```python
from build123d import *

# Parameters (mm, degrees)
BASE_BLOCK_SKETCH_W              = 200
BASE_BLOCK_SKETCH_H              = 160
BASE_BLOCK_DEPTH                 = 50
BEARING_HOUSING_DEPTH            = 50
BASE_RELIEF_CUT_SKETCH_W         = 100
BASE_RELIEF_CUT_SKETCH_H         = 100
BASE_RELIEF_CUT_DEPTH            = 50
BEARING_BORE_SKETCH_R            = 65
BEARING_BORE_DEPTH_35_DEPTH      = 35
FORK_SLOT_DEPTH                  = 200
UPPER_ARM_DEPTH                  = 30
UPPER_START                      = -30
UPPER_ARM_LUG_DEPTH              = 30
UPPER_LUG_COUNTERBORE_SKETCH_R   = 18
UPPER_LUG_COUNTERBORE_36X5_DEPTH = 5
UPPER_LUG_HOLE_SKETCH_R          = 7
UPPER_LUG_HOLE_14_DEPTH          = 50
UPPER_START_2                    = -5
UPPER_ARM_COUNTERBORE_SKETCH_R   = 18
UPPER_ARM_COUNTERBORE_36X5_DEPTH = 5
UPPER_START_3                    = -50
UPPER_ARM_HOLE_SKETCH_R          = 7
UPPER_ARM_HOLE_14_DEPTH          = 50
LOWER_ARM_DEPTH                  = 30
LOWER_START                      = -30
LOWER_ARM_LUG_DEPTH              = 30
LOWER_ARM_COUNTERBORE_SKETCH_R   = 18
LOWER_ARM_COUNTERBORE_36X5_DEPTH = 5
LOWER_ARM_HOLE_SKETCH_R          = 10
LOWER_ARM_HOLE_20_DEPTH          = 40
CROSS_HOLE_SKETCH_R              = 10
CROSS_HOLE_20_DEPTH              = 160
LOWER_START_2                    = -5
LOWER_LUG_COUNTERBORE_SKETCH_R   = 18
LOWER_LUG_COUNTERBORE_36X5_DEPTH = 5
LOWER_LUG_HOLE_SKETCH_R          = 10
LOWER_LUG_HOLE_20_DEPTH          = 30
SHAFT_BORE_SKETCH_R              = 25
SHAFT_BORE_50_DEPTH              = 30


with BuildPart() as part:
    # Base Block Sketch → Base Block (new body)
    with BuildSketch(Plane.XY):
        with Locations((100, 80)):
            Rectangle(BASE_BLOCK_SKETCH_W, BASE_BLOCK_SKETCH_H)
    extrude(amount=BASE_BLOCK_DEPTH)

    # Bearing Housing Sketch → Bearing Housing (add)
    with BuildSketch(Plane.XY.offset(50)):
        with BuildLine():
            Line((0, 160), (0, 0))
            ThreePointArc((0, 0), (-80, 80), (0, 160))
        make_face()
    extrude(amount=-BEARING_HOUSING_DEPTH)

    # Base Relief Cut Sketch → Base Relief Cut (cut)
    with BuildSketch(Plane.XY.offset(50)):
        with Locations((150, 80)):
            Rectangle(BASE_RELIEF_CUT_SKETCH_W, BASE_RELIEF_CUT_SKETCH_H)
    extrude(amount=-BASE_RELIEF_CUT_DEPTH, mode=Mode.SUBTRACT)

    # Bearing Bore Sketch → Bearing Bore Depth 35 (cut)
    with BuildSketch(Plane.XY.offset(50)):
        with Locations((0, 80)):
            Circle(BEARING_BORE_SKETCH_R)
    extrude(amount=-BEARING_BORE_DEPTH_35_DEPTH, mode=Mode.SUBTRACT)

    # Fork Slot Sketch → Fork Slot (cut)
    with BuildSketch(Plane(origin=(100, 0, 0), x_dir=(0, 0, -1), z_dir=(1, 0, 0))):
        Polygon((-50, 80), (-50, 90), (-35, 90), (-35, 70), (-50, 70), align=None)
    extrude(amount=-FORK_SLOT_DEPTH, mode=Mode.SUBTRACT)

    # Upper Arm Sketch → Upper Arm (add)
    with BuildSketch(Plane.XZ):
        with BuildLine():
            Line((125, 0), (100, 0))
            Line((100, 0), (75, 0))
            Line((75, 0), (75, -36.5))
            ThreePointArc((75, -36.5), (100, -61.5), (125, -36.5))
            Line((125, -36.5), (125, 0))
        make_face()
    extrude(amount=-UPPER_ARM_DEPTH)

    # Upper Arm Lug Sketch → Upper Arm Lug (add)
    with BuildSketch(Plane(origin=(0, 160, 0), x_dir=(1, 0, 0), z_dir=(0, 1, 0)).offset(UPPER_START)):
        with BuildLine():
            Line((75, 36.5), (75, 0))
            Line((75, 0), (125, 0))
            Line((125, 0), (125, 36.5))
            ThreePointArc((125, 36.5), (100, 61.5), (75, 36.5))
        make_face()
    extrude(amount=UPPER_ARM_LUG_DEPTH)

    # Upper Lug Counterbore Sketch → Upper Lug Counterbore Ø36x5 (cut)
    with BuildSketch(Plane(origin=(0, 160, 0), x_dir=(1, 0, 0), z_dir=(0, 1, 0))):
        with Locations(Location((100, 36.5, 0), (0, 0, 270))):
            Circle(UPPER_LUG_COUNTERBORE_SKETCH_R)
    extrude(amount=-UPPER_LUG_COUNTERBORE_36X5_DEPTH, mode=Mode.SUBTRACT)

    # Upper Lug Hole Sketch → Upper Lug Hole Ø14 (cut)
    with BuildSketch(Plane(origin=(0, 155, 0), x_dir=(1, 0, 0), z_dir=(0, 1, 0))):
        with Locations(Location((100, 36.5, 0), (0, 0, 270))):
            Circle(UPPER_LUG_HOLE_SKETCH_R)
    extrude(amount=-UPPER_LUG_HOLE_14_DEPTH, mode=Mode.SUBTRACT)

    # Upper Arm Counterbore Sketch → Upper Arm Counterbore Ø36x5 (cut)
    with BuildSketch(Plane.XZ.offset(UPPER_START_2)):
        with Locations(Location((100, -36.5, 0), (0, 0, 90))):
            Circle(UPPER_ARM_COUNTERBORE_SKETCH_R)
    extrude(amount=UPPER_ARM_COUNTERBORE_36X5_DEPTH, mode=Mode.SUBTRACT)

    # Upper Arm Hole Sketch → Upper Arm Hole Ø14 (cut)
    with BuildSketch(Plane.XZ.offset(-5).offset(UPPER_START_3)):
        with Locations(Location((100, -36.5, 0), (0, 0, 90))):
            Circle(UPPER_ARM_HOLE_SKETCH_R)
    extrude(amount=UPPER_ARM_HOLE_14_DEPTH, mode=Mode.SUBTRACT)

    # Lower Arm Sketch → Lower Arm (add)
    with BuildSketch(Plane.XZ):
        with BuildLine():
            Line((225, 25), (200, 25))
            Line((200, 25), (200, 50))
            ThreePointArc((200, 50), (182.32233047, 7.32233047), (225, 25))
        make_face()
    extrude(amount=-LOWER_ARM_DEPTH)

    # Lower Arm Lug Sketch → Lower Arm Lug (add)
    with BuildSketch(Plane(origin=(0, 160, 0), x_dir=(1, 0, 0), z_dir=(0, 1, 0)).offset(LOWER_START)):
        with BuildLine():
            Line((200, -25), (225, -25))
            ThreePointArc((225, -25), (217.67766953, -7.32233047), (200, 0))
            Line((200, 0), (200, -25))
        make_face()
    extrude(amount=LOWER_ARM_LUG_DEPTH)

    # Lower Arm Counterbore Sketch → Lower Arm Counterbore Ø36x5 (cut)
    with BuildSketch(Plane.XZ):
        with Locations((200, 25)):
            Circle(LOWER_ARM_COUNTERBORE_SKETCH_R)
    extrude(amount=-LOWER_ARM_COUNTERBORE_36X5_DEPTH, mode=Mode.SUBTRACT)

    # Lower Arm Hole Sketch → Lower Arm Hole Ø20 (cut)
    with BuildSketch(Plane.XZ.offset(-5)):
        with Locations((200, 25)):
            Circle(LOWER_ARM_HOLE_SKETCH_R)
    extrude(amount=-LOWER_ARM_HOLE_20_DEPTH, mode=Mode.SUBTRACT)

    # Cross Hole Sketch → Cross Hole Ø20 (cut)
    with BuildSketch(Plane.XZ.offset(-5)):
        with Locations(Location((100, -36.5, 0), (0, 0, 270))):
            Circle(CROSS_HOLE_SKETCH_R)
    extrude(amount=-CROSS_HOLE_20_DEPTH, mode=Mode.SUBTRACT)

    # Lower Lug Counterbore Sketch → Lower Lug Counterbore Ø36x5 (cut)
    with BuildSketch(Plane(origin=(0, 160, 0), x_dir=(1, 0, 0), z_dir=(0, 1, 0)).offset(LOWER_START_2)):
        with Locations((200, -25)):
            Circle(LOWER_LUG_COUNTERBORE_SKETCH_R)
    extrude(amount=LOWER_LUG_COUNTERBORE_36X5_DEPTH, mode=Mode.SUBTRACT)

    # Lower Lug Hole Sketch → Lower Lug Hole Ø20 (cut)
    with BuildSketch(Plane(origin=(0, 160, 0), x_dir=(1, 0, 0), z_dir=(0, 1, 0)).offset(LOWER_START)):
        with Locations((200, -25)):
            Circle(LOWER_LUG_HOLE_SKETCH_R)
    extrude(amount=LOWER_LUG_HOLE_20_DEPTH, mode=Mode.SUBTRACT)

    # Shaft Bore Sketch → Shaft Bore Ø50 (cut)
    with BuildSketch(Plane.XY.offset(15)):
        with Locations((0, 80)):
            Circle(SHAFT_BORE_SKETCH_R)
    extrude(amount=-SHAFT_BORE_50_DEPTH, mode=Mode.SUBTRACT)


solid = part.part
```
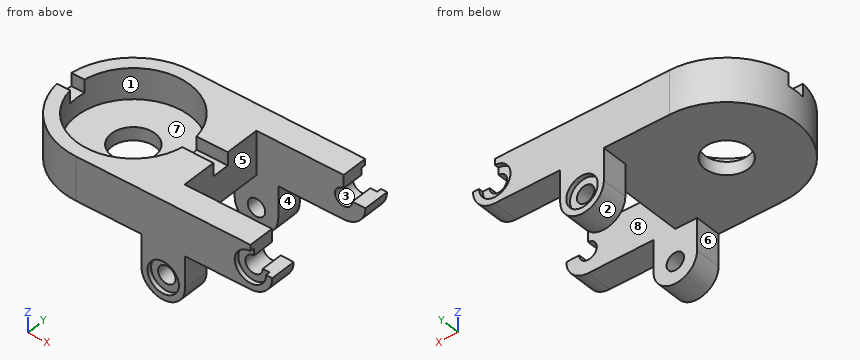
Part model, mm, in its own coordinate system. Face numbers are marked on the shaded views. A direction names the side the tool comes from. Round coordinates to 2 decimals unless told otherwise and drop trailing zeros. Order: outer loops, then holes, each group sorted by start corner. A loop starts at its lowest first (then second) coordinate and runs counter-clockwise, first axis right, second up. Notation, with made-up numbers: M 12,7 L 28,7 A23 ccw 28,22 Z; hole C -12,20 d2. An arc over 180 degrees is marked long. Put each result on its own line as item: value. Start each with the question number.
1. Slice it at B-B on x = 171. List the corners of the cut face in (y, z), then the cut area to 3 significant figures.
2. Slice it at C-C on z = 29.5. List the corners of the cut face in (x, y), then the cut area to 3 significant figures.
3. Slice it at D-D on y = 110. List the corners of the cut face in (x, z), then the cut area to 3 significant figures.
4. Drop flat-ended pins along their axis: pin 1 (4 mm diameter, centred on x = -37.5, y = 98.5, fed in from -Z); pin 2 (7.5 mm diameter, centred on x = 215.5, y = 13, fed in from +Z); pin 3 (2 mm diameter, centred on y = 18.5, z = -18, fed in from +X). Give the stop position or say it passes through.
5. Slice it at A-A on y = 80. List the corners of the cut face in (x, z).
6. Tool access for the marked faces 5, 6, 7 and 8: list every direction of +Z, -Z, +X, -X, +Y, -Y with a clear straight run to the whole face (end or side of a thin tool).
7. Drill centre lines: probe 1 along Z at (x, y) = (99.5, 28) (1 decimal); probe 2 along Z at (x, y) = (100, 2); probe 3 along X at (y, z) = (1.25, -36.5). Where is each one in solid material? Low to high. Write a range as [from, to].
8. Two-plate mould, pull along X, no slides. Class the marked faces 1, 2, 3 and 4: +X half, -X half, draft (parallel to the pull), parting line (faces both ways), or undercut.
Findings:
1. outline: M 0,0 L 30,0 L 30,50 L 0,50 Z; M 130,0 L 160,0 L 160,50 L 130,50 Z
1. area: 3,000 mm2
2. outline: M 0,0 L 182.57,0 L 182.57,5 L 191.07,5 L 191.07,30 L 100,30 L 100,130 L 191.07,130 L 191.07,155 L 182.57,155 L 182.57,160 L 0,160 A80 ccw Z; hole C 0,80 d130
2. area: 18,200 mm2
3. outline: M -74.16,0 L 100,0 L 100,50 L 57.66,50 L 57.66,15 L -57.66,15 L -57.66,50 L -74.16,50 Z
3. area: 4,670 mm2
4. pin 1: z = 0
4. pin 2: z = 25
4. pin 3: x = 125
5. outline: M -80,0 L -25,0 L -25,15 L -65,15 L -65,35 L -80,35 Z; M 25,0 L 100,0 L 100,35 L 65,35 L 65,15 L 25,15 Z
6. face 5: +Z, -Z, +X
6. face 6: -Z, -X, +Y, -Y
6. face 7: +Z
6. face 8: -Z, +X
7. probe 1: [-61.5, -46.5], [-26.5, 50]
7. probe 2: [-61.5, -54.5], [-18.5, 50]
7. probe 3: [75, 82], [118, 125]
8. face 1: undercut
8. face 2: parting line
8. face 3: undercut
8. face 4: +X half
